Geometry: see drawing. Coordinates: mm, zero at the bounding-box minimum. A direction names the side the tool comes from. Round coordinates to 2 decimals unless told otherwise and drop trailing zeros. Order: outer loops, then holes, each group sorted by start corner. A loop starts at its lowest first (then second) coordinate and runs counter-clockwise, first axis right, second up. Notation, with made-up numbers: (66, -12) -> (125, -12) arc R8 cw to (125, 1) -> close; hole circle Ø10 at (54, -14). An arc over 180 degrees is marked (long way). Write item = value, one per line. Start each with the question number.
(1) Ray query, line 1 (Y direction, x = 10, z = 15); line 2 (X direction, y = 68, z = 8.75); line 3 (Y direction, x = 7, z = 8.25). Return the intervals inside material, ascending.
(2) Reachability of the marked faces 1 and 2 from +Z, -Z, +X, -X, +Y, -Y: full face, straight path, thin tool, end or side. Return the list, or none.
(3) Cut plane B-B on y = 66. Return the cut outline in (x, z), then the cut area to 3 significant figures.
(4) Contact query for a flat-ended pin moving along its axis: pin 1 Ø10 at (y, z) = (65.5, 8.5) entering from -X. Output: stop coordinate, or through.
(5) Cut plane A-A on z = 13.75. Return the cut outline in (x, y).
(6) Draft query along Y for the marked faces 3, 4 and 5. Return one class per face: released by +Y, released by -Y, zero draft, split by the parting line, or undercut.
(7) Cut plane C-C on y = 91. Return the cut outline in (x, z), then the cut area to 3 significant figures.
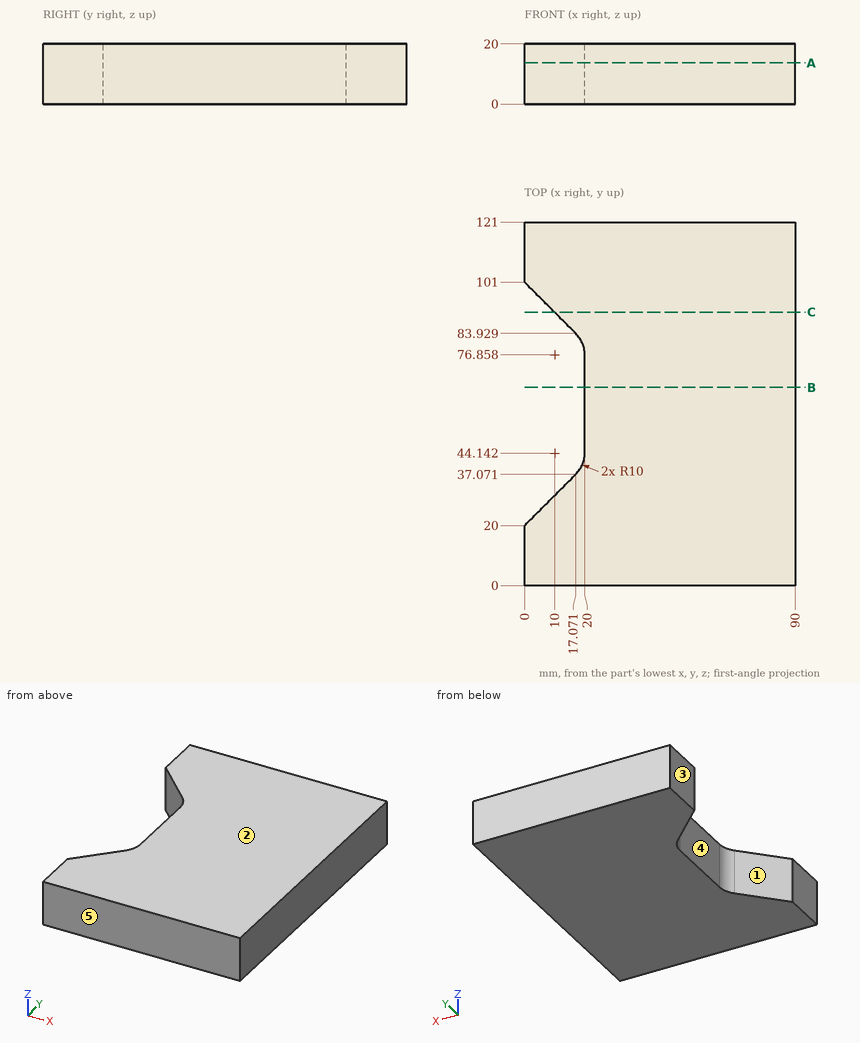
Evaluation:
q1.line_1 = 0 to 30, 91 to 121
q1.line_2 = 20 to 90
q1.line_3 = 0 to 27, 94 to 121
q2.face_1 = +Z, -Z, -X
q2.face_2 = +Z, +X, -X, +Y, -Y
q3.outline = (20, 0) -> (90, 0) -> (90, 20) -> (20, 20) -> close
q3.area = 1,400 mm^2
q4.pin_1 = 20
q5.outline = (0, 0) -> (90, 0) -> (90, 121) -> (0, 121) -> (0, 101) -> (17.07, 83.93) arc R10 cw to (20, 76.86) -> (20, 44.14) arc R10 cw to (17.07, 37.07) -> (0, 20) -> close
q6.face_3 = zero draft
q6.face_4 = undercut
q6.face_5 = released by -Y
q7.outline = (10, 0) -> (90, 0) -> (90, 20) -> (10, 20) -> close
q7.area = 1,600 mm^2
